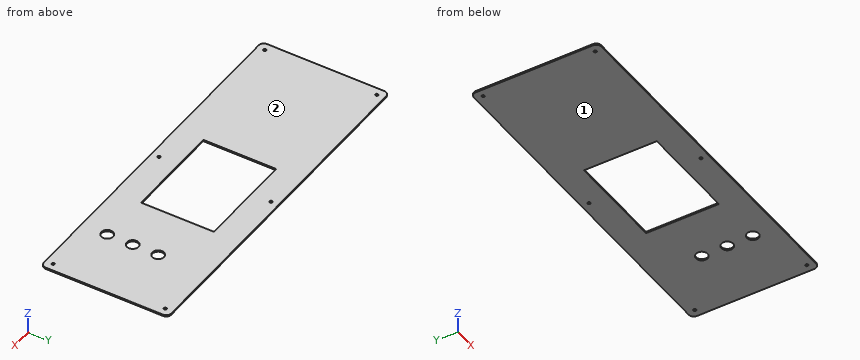
from build123d import *

# Parameters (mm, degrees)
SKETCH_1_W                  = 690
SKETCH_1_H                  = 250
EXTRUDE_1_DEPTH             = 1.5
SKETCH_2_W                  = 194
SKETCH_2_H                  = 143
CUT_EXTRUDE_1_DEPTH         = 6
SKETCH_3_R                  = 11.5
CUT_EXTRUDE_2_DEPTH         = 6
FILLET_1_R                  = 10
HOLE_WIZARD_5_5_5_5_1_D     = 5.5
HOLE_WIZARD_5_5_5_5_1_DEPTH = 10
HOLE_WIZARD_5_5_5_5_1_TIP   = 1.652366702


with BuildPart() as part:
    # 草图1 → 凸台-拉伸1 (new, symmetric)
    with BuildSketch(Plane.XY):
        Rectangle(SKETCH_1_W, SKETCH_1_H)
    extrude(amount=EXTRUDE_1_DEPTH, both=True)

    # 草图2 → 切除-拉伸1 (cut)
    with BuildSketch(Plane.XY.offset(1.5)):
        with Locations((20, 0)):
            Rectangle(SKETCH_2_W, SKETCH_2_H)
    extrude(amount=-CUT_EXTRUDE_1_DEPTH, mode=Mode.SUBTRACT)

    # 草图3 → 切除-拉伸2 (cut)
    with BuildSketch(Plane.XY.offset(1.5)):
        with Locations((217, -25)):
            Circle(SKETCH_3_R)
        with Locations((217, -75)):
            Circle(SKETCH_3_R)
        with BuildLine():
            ThreePointArc((205.992928436, 28.33082206), (219.353810017, 13.74346508), (225.750187968, 32.462185372))
            ThreePointArc((225.750187968, 32.462185372), (214.646189983, 36.25653492), (205.992928436, 28.33082206))
        make_face()
    extrude(amount=-CUT_EXTRUDE_2_DEPTH, mode=Mode.SUBTRACT)

    # 圆角1
    fillet_1_edges = [part.edges().sort_by_distance(p)[0] for p in [
        (345, -125, 0),
        (-345, -125, 0),
        (-345, 125, 0),
        (345, 125, 0),
    ]]
    fillet(fillet_1_edges, radius=FILLET_1_R)

    # Ø5.5 (5.5) 直径孔1
    with Locations(Plane.XY.offset(1.5)):
        with Locations((-330, 110), (0, 110), (330, 110), (330, -110), (0, -110), (-330, -110)):
            Hole(HOLE_WIZARD_5_5_5_5_1_D / 2, depth=HOLE_WIZARD_5_5_5_5_1_DEPTH)
            with Locations((0, 0, -(HOLE_WIZARD_5_5_5_5_1_DEPTH + HOLE_WIZARD_5_5_5_5_1_TIP / 2))):  # 118° drill point
                Cone(0, HOLE_WIZARD_5_5_5_5_1_D / 2, HOLE_WIZARD_5_5_5_5_1_TIP, mode=Mode.SUBTRACT)


solid = part.part
Could you check a few things on this model? Use its own coordinates, in mm. Face numbers are marked on the shaded views. Coordinates: 2 decimals unless noted, no trailing zeros. Write each loop counter-clockwise with the first axis right and the second up, starting at its lowest first coordinate (ties: lowest second). Pieces come first, ordered by that corner, then holes. Notation, with made-up numbers: (10.5, 61.25) - (61.5, 61.25) arc R36 ccw to (61.5, 98.25) - close; hole circle Ø9 at (14, 40). An arc over 180 degrees is marked (long way). Put each result on its own line as item: value. Start each with the question number.
Q1. I want a section at D-D on x = 16. Write out the boundary of the cut face in (y, z), plus the area to 3 significant figures.
Q2. I want a section at C-C on z = 0.45. Count the separate pieces of the cut face and the enclosed holes in it, plus the area to 3 significant figures.
Q3. Thinking about a two-plate mould opening in Z: for the marked faces 1 and 2, which applies, pulls with the +Z half, pulls with the -Z half, needs draft (parallel to the pull), parting line crosses it, or undercut?
Q4. I want a section at B-B on y = -25. Write out the boundary of the cut face in (x, z), plus the area to 3 significant figures.
Q5. Please list where these lines run through material, in increasing order: L1, parallel to Y at x = 330, z = -0.7; L2, parallel to Y at x = 0, z = -0.7; L3, parallel to Y at x = 46, z = 0.2.
Q6. I want a section at A-A on x = 217. Write out the boundary of the cut face in (y, z).
Checks:
1. outline: (-125, -1.5) - (-71.5, -1.5) - (-71.5, 1.5) - (-125, 1.5) - close; (71.5, -1.5) - (125, -1.5) - (125, 1.5) - (71.5, 1.5) - close
1. area: 321 mm²
2. separate pieces: 1
2. enclosed holes: 10
2. area: 143,000 mm²
3. face 1: pulls with the -Z half
3. face 2: pulls with the +Z half
4. outline: (-345, -1.5) - (-77, -1.5) - (-77, 1.5) - (-345, 1.5) - close; (117, -1.5) - (205.5, -1.5) - (205.5, 1.5) - (117, 1.5) - close; (228.5, -1.5) - (345, -1.5) - (345, 1.5) - (228.5, 1.5) - close
4. area: 1,420 mm²
5. L1: -125 to -112.75, -107.25 to 107.25, 112.75 to 125
5. L2: -125 to -112.75, -107.25 to -71.5, 71.5 to 107.25, 112.75 to 125
5. L3: -125 to -71.5, 71.5 to 125
6. outline: (-125, -1.5) - (-86.5, -1.5) - (-86.5, 1.5) - (-125, 1.5) - close; (-63.5, -1.5) - (-36.5, -1.5) - (-36.5, 1.5) - (-63.5, 1.5) - close; (-13.5, -1.5) - (13.5, -1.5) - (13.5, 1.5) - (-13.5, 1.5) - close; (36.5, -1.5) - (125, -1.5) - (125, 1.5) - (36.5, 1.5) - close
